Model file for the job. Use its own axes, mm. Coordinates: 2 decimals unless noted, no trailing zeros. Order: outer loops, then holes, each group sorted by start corner. A loop starts at its lowest first (then second) coordinate and runs counter-clockwise, first axis right, second up. Notation, with made-up numbers: (39, 61.25) -> (44, 61.25) arc R33 ccw to (44, 91.25) -> close; hole circle Ø6 at (55.5, 47). An arc over 180 degrees is marked (long way). Write item = value, one per line. Start each with the question number.
Q1. Wall check: line 1 (Z direction, x = 60, y = 6.75); line 2 (X direction, y = 7, z = -12); line 3 (Z direction, x = 57.5, y = 3). Give the ranges that are in metal, low to high. Write a range as from..to.
Q2. Cut at A-A, the plane z = -188. List the corners of the cut face in (x, y), plus the area to 3 significant figures.
Q3. Cut at B-B, the plane x = 10. List the corners of the cut face in (y, z).
Q4. Flat gauge pin, fed straight in: pin 1 (6 mm diameter, centred on x = 60, z = -12, fed in from -Y). Where does the tip first touch, or does it go through?
Q5. Mould opens along X. For faces 1 (the face through (61.6, 7.1, -185)), 2 (the face through (70, 7, -99)), 3 (the face through (35, 7, 0)) say: +X half, -X half, draft (parallel to the pull), parting line (faces both ways), or undercut.
from build123d import *

# Parameters (mm, degrees)
SKETCH1_W           = 70
SKETCH1_H           = 200
BOSS_EXTRUDE1_DEPTH = 14
M8_TAPPED_HOLE1_D   = 6.8


with BuildPart() as part:
    # Sketch1 → Boss-Extrude1 (new body)
    with BuildSketch(Plane(origin=(0, 0, 0), x_dir=(1, 0, 0), z_dir=(0, 1, 0))):
        with Locations((35, 100)):
            Rectangle(SKETCH1_W, SKETCH1_H)
    extrude(amount=BOSS_EXTRUDE1_DEPTH)

    # M8 Tapped Hole1 (through all)
    with Locations(Plane(origin=(0, 0, 0), x_dir=(-1, 0, 0), z_dir=(0, -1, 0))):
        with Locations((-60, 188), (-10, 188), (-10, 12), (-60, 12)):
            Hole(M8_TAPPED_HOLE1_D / 2)


solid = part.part
Here are the results:
q1.line_1 = -200..-191.4, -184.6..-15.4, -8.6..0
q1.line_2 = 0..6.6, 13.4..56.6, 63.4..70
q1.line_3 = -200..-190.3, -185.7..-14.3, -9.7..0
q2.outline = (0, 0) -> (6.6, 0) -> (6.6, 14) -> (0, 14) -> close; (13.4, 0) -> (56.6, 0) -> (56.6, 14) -> (13.4, 14) -> close; (63.4, 0) -> (70, 0) -> (70, 14) -> (63.4, 14) -> close
q2.area = 790 mm²
q3.outline = (0, -200) -> (14, -200) -> (14, -191.4) -> (0, -191.4) -> close; (0, -184.6) -> (14, -184.6) -> (14, -15.4) -> (0, -15.4) -> close; (0, -8.6) -> (14, -8.6) -> (14, 0) -> (0, 0) -> close
q4.pin_1 = through
q5.face_1 = undercut
q5.face_2 = +X half
q5.face_3 = draft
